CAD build for the part. Positions are in the model's coordinates, mm. A direction names the side the tool comes from. Round coordinates to 2 decimals unless told otherwise and drop trailing zeros. Loops run counter-clockwise (first coordinate to the right, second up) from the corner with the lowest first, then second, coordinate; pieces in that order, holes last. Notation, with made-up numbers: (-22.5, -33.5) -> (24.5, -33.5) arc R18 cw to (24.5, -22.5) -> close; hole circle Ø2 at (54, 45). An arc over 180 degrees is marked (long way). Answer as CSV lines item,"result".
```python
from build123d import *

# Parameters (mm, degrees)
SKETCH_1_W               = 180
SKETCH_1_H               = 180
EXTRUDE_1_DEPTH          = 41
SKETCH_2_R               = 75
EXTRUDE_2_DEPTH          = 15
SKETCH_3_R               = 63
CUT_EXTRUDE_1_DEPTH      = 13
SKETCH_4_W               = 6.5
SKETCH_4_H               = 5
CUT_EXTRUDE_2_REACH      = 136.347
CUT_EXTRUDE_2_END_RADIUS = 5.5626
SKETCH_9_R               = 3
CUT_EXTRUDE_3_REACH      = 141.054
SKETCH_10_R              = 8.5


with BuildPart() as part:
    # 草图1 → 凸台-拉伸1 (new body)
    with BuildSketch(Plane.XY):
        Rectangle(SKETCH_1_W, SKETCH_1_H)
    extrude(amount=EXTRUDE_1_DEPTH)

    # 草图2 → 凸台-拉伸2 (add)
    with BuildSketch(Plane.XY.offset(41)):
        Circle(SKETCH_2_R)
    extrude(amount=EXTRUDE_2_DEPTH)

    # 草图3 → 切除-拉伸1 (cut)
    with BuildSketch(Plane.XY.offset(56)):
        Circle(SKETCH_3_R)
    extrude(amount=-CUT_EXTRUDE_1_DEPTH, mode=Mode.SUBTRACT)

    # 草图4 → 切除-旋转1 (revolve, cut)
    with BuildSketch(Plane(origin=(0, 0, 0), x_dir=(0, 0, -1), z_dir=(1, 0, 0)), mode=Mode.PRIVATE) as cut_revolve_1_sk:
        with Locations((-49.25, 72.5)):
            Rectangle(SKETCH_4_W, SKETCH_4_H)
    revolve(cut_revolve_1_sk.sketch.rotate(Axis((0, 0, 56), (0, 0, -1)), 90), axis=Axis((0, 0, 56), (0, 0, -1)), mode=Mode.SUBTRACT)

    # 草图6 → 1/4 NPT 螺纹孔1 (revolve, cut)
    with BuildSketch(Plane(origin=(0, 90, 23), x_dir=(0, 0, 1), z_dir=(1, 0, 0))):
        Polygon((0, 0), (0, 36.342347279), (5.5626, 33), (5.5626, 10.02), (5.943676082, 10.02), (6.2436883, 0), align=None)
    revolve(axis=Axis((0, 96.35, 23), (0, -1, 0)), mode=Mode.SUBTRACT)

    # 草图8 → 切除-旋转2 (revolve, cut)
    with BuildSketch(Plane(origin=(0, 0, 0), x_dir=(1, 0, 0), z_dir=(0, 1, 0))):
        Polygon((0, -56), (22.5, -56), (22.5, -40), (25, -40), (25, -33.5), (20, -33.5), (20, -28.5), (22.5, -28.5), (22.5, -22), (20, -22), (20, -17), (22.5, -17), (22.5, -13), (20, -13), (20, -8), (22.5, -8), (22.5, -4), (20, -4), (20, 0), (0, 0), align=None)
    revolve(axis=Axis((0, 0, 56), (0, 0, -1)), mode=Mode.SUBTRACT)

    # 切除-拉伸2: up to this cylinder (the profile starts outside it)
    cut_extrude_2_end = Plane(origin=(0, 60, 23), z_dir=(0, 1, 0)) * Cylinder(CUT_EXTRUDE_2_END_RADIUS, 284.8192, mode=Mode.PRIVATE)
    # 草图9 → 切除-拉伸2 (cut, up to the surface)
    with BuildSketch(Plane.XY.offset(43), mode=Mode.PRIVATE) as cut_extrude_2_sk1:
        with Locations(Location((0, 60, 0), (0, 0, 270))):
            Circle(SKETCH_9_R)
    cut_extrude_2_tool1 = extrude(cut_extrude_2_sk1.sketch, amount=-CUT_EXTRUDE_2_REACH, mode=Mode.PRIVATE) - cut_extrude_2_end
    add(cut_extrude_2_tool1.solids().sort_by_distance((0, 60, 43))[0], mode=Mode.SUBTRACT)

    # 草图10 → 切除-拉伸3 (cut, up to next)
    with BuildSketch(Plane(origin=(0, 0, 0), x_dir=(-1, 0, 0), z_dir=(0, 0, -1)), mode=Mode.PRIVATE) as cut_extrude_3_sk1:
        with Locations((-70, 70)):
            Circle(SKETCH_10_R)
    cut_extrude_3_tool1 = extrude(cut_extrude_3_sk1.sketch, amount=-CUT_EXTRUDE_3_REACH, mode=Mode.PRIVATE) & part.part
    # 草图10 → 切除-拉伸3 (cut, up to next)
    with BuildSketch(Plane(origin=(0, 0, 0), x_dir=(-1, 0, 0), z_dir=(0, 0, -1)), mode=Mode.PRIVATE) as cut_extrude_3_sk2:
        with Locations((70, 70)):
            Circle(SKETCH_10_R)
    cut_extrude_3_tool2 = extrude(cut_extrude_3_sk2.sketch, amount=-CUT_EXTRUDE_3_REACH, mode=Mode.PRIVATE) & part.part
    # 草图10 → 切除-拉伸3 (cut, up to next)
    with BuildSketch(Plane(origin=(0, 0, 0), x_dir=(-1, 0, 0), z_dir=(0, 0, -1)), mode=Mode.PRIVATE) as cut_extrude_3_sk3:
        with Locations((70, -70)):
            Circle(SKETCH_10_R)
    cut_extrude_3_tool3 = extrude(cut_extrude_3_sk3.sketch, amount=-CUT_EXTRUDE_3_REACH, mode=Mode.PRIVATE) & part.part
    # 草图10 → 切除-拉伸3 (cut, up to next)
    with BuildSketch(Plane(origin=(0, 0, 0), x_dir=(-1, 0, 0), z_dir=(0, 0, -1)), mode=Mode.PRIVATE) as cut_extrude_3_sk4:
        with Locations((-70, -70)):
            Circle(SKETCH_10_R)
    cut_extrude_3_tool4 = extrude(cut_extrude_3_sk4.sketch, amount=-CUT_EXTRUDE_3_REACH, mode=Mode.PRIVATE) & part.part
    add(cut_extrude_3_tool1.solids().sort_by_distance((70, 70, 0))[0], mode=Mode.SUBTRACT)
    add(cut_extrude_3_tool2.solids().sort_by_distance((-70, 70, 0))[0], mode=Mode.SUBTRACT)
    add(cut_extrude_3_tool3.solids().sort_by_distance((-70, -70, 0))[0], mode=Mode.SUBTRACT)
    add(cut_extrude_3_tool4.solids().sort_by_distance((70, -70, 0))[0], mode=Mode.SUBTRACT)


solid = part.part
```
Q1. Two-plate mould, pull along Y, no slides. Class faces 5 (the flat face through (-17, 61, 56)), 6 (the flat face through (-11, -17, 33.5)), 7 (the conical face through (0.37, 54.238, 23.892)): pulls with the +Y half, pulls with the -Y half, needs draft (parallel to the pull), parting line crosses it, or undercut.
Results:
face 5,"needs draft"
face 6,"undercut"
face 7,"pulls with the +Y half"
Q2. Slice it at A-A, the plane y = 66. Give the cut face in (x, z), and give its area (3 significant figures).
Results:
outline,"(-90, 0) -> (-77.5, 0) -> (-77.5, 41) -> (-90, 41) -> close; (-62.5, 0) -> (62.5, 0) -> (62.5, 41) -> (35.62, 41) -> (35.62, 46) -> (23.32, 46) -> (23.32, 52.5) -> (35.62, 52.5) -> (35.62, 56) -> (-35.62, 56) -> (-35.62, 52.5) -> (-23.32, 52.5) -> (-23.32, 46) -> (-35.62, 46) -> (-35.62, 41) -> (-62.5, 41) -> close; (77.5, 0) -> (90, 0) -> (90, 41) -> (77.5, 41) -> close; hole circle Ø11.13 at (0, 23)"
area,"6,960 mm2"
Q3. Drop flat-ended pins along their axis: pin 1 Ø13.5 at (x, y) = (3.5, 7) entering from +Z; pin 2 Ø3.5 at (x, z) = (1.5, 21.5) entering from +Y; pin 3 Ø12 at (y, z) = (-41.5, 48.5) entering from -X; pin 4 Ø4 at (x, y) = (44.5, 70) entering from +Z. Give the stop position or say it passes through.
Results:
pin 1,"through"
pin 2,"y = 55.98"
pin 3,"x = -65.77"
pin 4,"z = 41"
Q4. Probe L1, parallel to Y at x = -70, z = 10; L2, parallel to Z at x = -71, y = -10; L3, parallel to X at y = 0, z = 23.75. List the from-to ranges inside material, lowest first. Write a range as [from, to].
Results:
L1,"[-90, -78.5], [-61.5, 61.5], [78.5, 90]"
L2,"[0, 46], [52.5, 56]"
L3,"[-90, -22.5], [22.5, 90]"
Q5. Slice it at B-B, the plane y = 37.5. Give the cut face in (x, z), and give its area (3 significant figures).
Results:
outline,"(-90, 0) -> (90, 0) -> (90, 41) -> (64.95, 41) -> (64.95, 46) -> (59.11, 46) -> (59.11, 52.5) -> (64.95, 52.5) -> (64.95, 56) -> (50.62, 56) -> (50.62, 43) -> (-50.62, 43) -> (-50.62, 56) -> (-64.95, 56) -> (-64.95, 52.5) -> (-59.11, 52.5) -> (-59.11, 46) -> (-64.95, 46) -> (-64.95, 41) -> (-90, 41) -> close"
area,"7,940 mm2"
Q6. Tool access for faces 1 (the cylindrical face through (10.382, 19.961, 14.972)), 2 (the cylindrical face through (-8.201, 62.464, 49.591)), 3 (the cylindrical face through (-0.245, 68.651, 17.443)), 4 (the flat face through (90, -1, 20)): list every direction of +Z, -Z, +X, -X, +Y, -Y with a clear straight run to the whole face (end or side of a thin tool).
Results:
face 1,"none"
face 2,"+Z"
face 3,"+Y"
face 4,"+Z, -Z, +X, +Y, -Y"
